from build123d import *

# Parameters (mm, degrees)
BRACKET_BODY_DEPTH                = 11
FORK_SLOT_SKETCH_W                = 36.5
FORK_SLOT_SKETCH_H                = 8
FORK_SLOT_8MM_DEPTH               = 77.995129716
MOUNTING_HOLE_CBORE_8_D           = 8
MOUNTING_HOLE_CBORE_8_CBORE_D     = 12
MOUNTING_HOLE_CBORE_8_CBORE_DEPTH = 4
CROSS_HOLE_SKETCH_R               = 4
CROSS_HOLE_8_DEPTH                = 80.317400361
CROSS_HOLE_CHAMFER_1MM_SIZE       = 1


with BuildPart() as part:
    # Bracket Profile Sketch → Bracket Body (new, symmetric)
    with BuildSketch(Plane.XY):
        with BuildLine():
            Line((0, 0), (32, 0))
            Line((32, 0), (49.5, 0))
            ThreePointArc((49.5, 0), (59.208203932, 4.946576972), (60.912678196, 15.708203932))
            Line((60.912678196, 15.708203932), (52.06873868, 42.927050983))
            ThreePointArc((52.06873868, 42.927050983), (50.978924888, 44.427050983), (49.215569131, 45))
            Line((49.215569131, 45), (41, 45))
            Line((41, 45), (41, 37.5))
            Line((41, 37.5), (43.5, 37.5))
            Line((43.5, 37.5), (43.5, 19.95706006))
            Line((43.5, 19.95706006), (25, 15))
            Line((25, 15), (0, 15))
            Line((0, 15), (0, 0))
        make_face()
    extrude(amount=BRACKET_BODY_DEPTH, both=True)

    # Fork Slot Sketch → Fork Slot 8mm (cut, through all)
    with BuildSketch(Plane(origin=(0, 0, 0), x_dir=(1, 0, 0), z_dir=(0, 1, 0))):
        with Locations((43.25, 0)):
            Rectangle(FORK_SLOT_SKETCH_W, FORK_SLOT_SKETCH_H)
    extrude(amount=FORK_SLOT_8MM_DEPTH, mode=Mode.SUBTRACT)

    # Mounting Hole CBore Ø8 (through all)
    with Locations(Plane(origin=(12.5, 15, 0), x_dir=(0, 0, 1), z_dir=(0, 1, 0))):
        with Locations((0, 0)):
            CounterBoreHole(MOUNTING_HOLE_CBORE_8_D / 2, MOUNTING_HOLE_CBORE_8_CBORE_D / 2, MOUNTING_HOLE_CBORE_8_CBORE_DEPTH)

    # Cross Hole Sketch → Cross Hole Ø8 (cut, through all)
    with BuildSketch(Plane.XY.offset(11)):
        with Locations((32, 7.5)):
            Circle(CROSS_HOLE_SKETCH_R)
    extrude(amount=-CROSS_HOLE_8_DEPTH, mode=Mode.SUBTRACT)

    # Cross Hole Chamfer 1mm
    cross_hole_chamfer_1mm_edges = [part.edges().sort_by_distance(p)[0] for p in [
        (28, 7.5, -11),
        (28, 7.5, 11),
    ]]
    chamfer(cross_hole_chamfer_1mm_edges, length=CROSS_HOLE_CHAMFER_1MM_SIZE)


solid = part.part
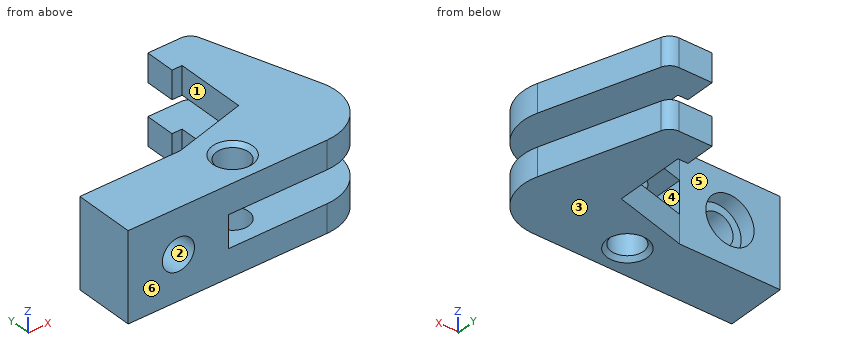
Can you work these out from the model? Positions are in its coordinate system, mm. Face numbers are marked on the shaded views. A direction names the side the tool comes from. Coordinates: 2 decimals unless noted, no trailing zeros. Loops run counter-clockwise (first coordinate to the right, second up) from the corner with the lowest first, then second, coordinate; pieces in that order, holes last. Notation, with made-up numbers: (63.25, 1.5) - (83.25, 1.5) arc R14 cw to (83.25, 14.5) - close; hole circle Ø10 at (-2.5, -32). An arc over 180 degrees is marked (long way). Answer as a JSON object with one key per item and string values. Group by question number.
Item 1: If we section it at C-C (y = 7.5): List the corners of the cut face in (x, z) for me.
Item 2: If we mould it in two halves opening along Z, with no side actions, what happens to the marked faces 1, 2 and 3? For each: released by +Z, released by -Z, zero draft, split by the parting line, or undercut.
Item 3: If we section it at B-B (z = 0): List the corners of the cut face in (x, y) for me, plus the area to 3 significant figures.
Item 4: For pin 1 (11 mm diameter, centred on x = 35.5, y = 27, fed in from -Z); pin 2 (2 mm diameter, centred on y = 32, z = -7, fed in from -X); pin 3 (13 mm diameter, centred on x = 12.5, z = 0, fed in from +Y); pin 4 (9 mm diameter, centred on x = 32, y = 7.5, fed in from +Z), each with a flat end and sliding along its axis, tell me the tip position at first contact or that it passes through.
Item 5: If I drill on L1, parallel to Z at x = 44.5, y = 2.5; L2, parallel to X at y = 13.35, z = 0; L3, parallel to X at y = 4.25, z = 0, over which ranges is the centre line in solid material (lowest first)? Write a range as from..to.
Item 6: If we section it at D-D (y = 27): List the corners of the cut face in (x, z) for me.
Item 7: If we section it at A-A (x = 12.5): List the corners of the cut face in (y, z) for me, plus the area to 3 significant figures.
Item 8: On a 3-axis mill with a long thin cutter (end or side, diameter ignored), from which of +Z, -Z, +X, -X, +Y, -Y can I reach the whole of each face in a straight line? I mean the marked faces 4, 5 and 6. Say none if no direction works.
Returned:
{
 "1": {"outline": "(0, -11) - (27, -11) - (28, -10) - (28, -4) - (25, -4) - (25, 4) - (28, 4) - (28, 10) - (27, 11) - (0, 11) - close; (36, -10) - (37, -11) - (60.62, -11) - (60.62, -4) - (36, -4) - close; (36, 4) - (60.62, 4) - (60.62, 11) - (37, 11) - (36, 10) - close; hole circle Ø8 at (12.5, 0)"},
 "2": {"face 1": "zero draft", "face 2": "undercut", "face 3": "released by -Z"},
 "3": {"outline": "(0, 0) - (8.5, 0) - (8.5, 11) - (6.5, 11) - (6.5, 15) - (0, 15) - close; (16.5, 0) - (25, 0) - (25, 15) - (18.5, 15) - (18.5, 11) - (16.5, 11) - close", "area": "239 mm²"},
 "4": {"pin 1": "passes through", "pin 2": "stops at x = 43.5", "pin 3": "stops at y = 15", "pin 4": "stops at z = 10.5"},
 "5": {"L1": "z = -11..-4, 4..11", "L2": "x = 0..6.5, 18.5..25", "L3": "x = 0..8.5, 16.5..25"},
 "6": {"outline": "(43.5, -11) - (57.24, -11) - (57.24, -4) - (43.5, -4) - close; (43.5, 4) - (57.24, 4) - (57.24, 11) - (43.5, 11) - close"},
 "7": {"outline": "(0, -11) - (15, -11) - (15, -6) - (11, -6) - (11, -4) - (0, -4) - close; (0, 4) - (11, 4) - (11, 6) - (15, 6) - (15, 11) - (0, 11) - close", "area": "194 mm²"},
 "8": {"face 4": "+X, +Y, -Y", "face 5": "+Z, -Z, -X, +Y", "face 6": "+Z, -Z, +X, -X, -Y"}
}
